Source: CAD feature listing. Evaluate the final solid. Frame: model axes, mm. A direction names the side the tool comes from. Round coordinates to 2 decimals unless told otherwise and drop trailing zeros. Write each loop counter-clockwise with the first axis right and the second up, starting at its lowest first coordinate (ties: lowest second). Pieces come first, ordered by that corner, then holes.
from build123d import *


with BuildPart() as part:
    # 草图1 → 旋转1 (revolve)
    with BuildSketch(Plane.XY, mode=Mode.PRIVATE) as revolve_1_sk:
        Polygon((0, 0), (2.5, 0), (5.951105222, 3), (5.951105222, 4), (2.5, 1), (2.5, 4), (0, 4), align=None)
    revolve(revolve_1_sk.sketch.rotate(Axis((-6.870284449, -15.5, 0), (1, 0, 0)), 90), axis=Axis((-6.870284449, -15.5, 0), (1, 0, 0)))


solid = part.part
1) Contact query for flat-ended pins moving along their axis: P1, Ø1, axis at y = -24.5, z = 12.5, coming from the +X side; P2, Ø1.5, axis at x = 3, z = 15, coming from the -Y side; P3, Ø3, axis at x = 2.5, y = -8.5, coming from the -Z side. Output: stop coordinate, or through.
Taken from the geometry:
P1: stops at x = 2.96
P2: stops at y = -28.6
P3: stops at z = -18.71
2) Section query B-B on z = 0. Return the cut outline in (x, y), then the cut area to 3 significant figures.
Taken from the geometry:
outline: (0, -35) - (2.5, -35) - (2.5, -32) - (5.95, -35) - (5.95, -34) - (2.5, -31) - (0, -31) - close; (0, 0) - (2.5, 0) - (5.95, 3) - (5.95, 4) - (2.5, 1) - (2.5, 4) - (0, 4) - close
area: 26.9 mm2
3) Pull-direction query (Y, two-part tool) for faces 3 (the face through (1.232, 3.536, -4.227)), 4 (the face through (0, -6.9, -13.1)), 5 (the face through (1.268, -30.868, -2.018)); classes: released by +Y, released by -Y, zero draft, split by the parting line, or undercut.
Taken from the geometry:
face 3: split by the parting line
face 4: zero draft
face 5: undercut
4) Section query A-A on y = -15.5. Return the cut outline in (x, z).
Taken from the geometry:
outline: (0, -19.5) - (2.5, -19.5) - (2.5, -16.5) - (5.95, -19.5) - (5.95, -18.5) - (2.5, -15.5) - (0, -15.5) - close; (0, 15.5) - (2.5, 15.5) - (5.95, 18.5) - (5.95, 19.5) - (2.5, 16.5) - (2.5, 19.5) - (0, 19.5) - close
5) Reachability of faces 1 (the face through (2.5, -24, 15)), 2 (the face through (5.951, -4, 15)) from +Z, -Z, +X, -X, +Y, -Y: full face, straight path, thin tool, end or side. Return the list, or none.
Taken from the geometry:
face 1: none
face 2: +Z, -Z, +X, +Y, -Y
6) Material intervals for line 1 (Y direction, x = 1.65, z = 0); line 2 (Y direction, x = 5.2, z = 15); line 3 (Z direction, x = 4.95, y = -30.5), sorted ascending.
Taken from the geometry:
line 1: y = -35 to -31, 0 to 4
line 2: y = -26.91 to -25.17, -5.83 to -4.09
line 3: z = -11.05 to -9.26, 9.26 to 11.05
7) Section query C-C on x = 4.8. Return the cut outline in (y, z), then the cut area to 3 significant figures.
Taken from the geometry:
outline: circle Ø37 at (-15.5, 0); hole circle Ø35 at (-15.5, 0)
area: 113 mm2
